Check sheet for the modelled part. Datum: model origin and axes. Units: mm. A direction names the side the tool comes from. Give positions to 0.01 mm unless a question says otherwise; leave off trailing zeros. Write each loop counter-clockwise with the first axis right and the second up, starting at its lowest first coordinate (ties: lowest second). Pieces come first, ordered by that corner, then holes. Notation, with made-up numbers: M 4,-33.5 L 39,-33.5 A27 cw 39,-16.5 Z; hole C 86,-31 d7. An arc over 180 degrees is marked long. Write item = value, one per line. Start each with the question number.
1) Mould release check, pull along Z, two halves, no side actions. Record for faces 1 (the cylindrical face through (48.89, -47.76, 69.79)), 2 (the cylindrical face through (-59.94, 2.64, 37.33)), 3 (the conical face through (-0.03, 60.74, 60.89)): released by +Z, released by -Z, zero draft, split by the parting line, or undercut.
2) Cross-section at C-C, the plane z = 76. Record the cut outline in (x, y).
3) Cross-section at B-B, the plane x = 75. Record the cut outline in (y, z), plus the area to 3 significant figures.
4) Cross-section at A-A, the plane z = 8. Record the cut outline in (x, y), plus the area to 3 significant figures.
5) Access from +Z, -Z, +X, -X, +Y, -Y to the whole of each face (thin tool, end or side, straight path). Record for faces 4 (the cylindrical face through (-48.89, 47.76, 69.79)), 5 (the cylindrical face through (-47.76, -48.89, 69.79)), 6 (the flat face through (46.5, 46.5, 55)), 7 (the cylindrical face through (55.946, 1.277, 74.154)).
6) Scan lines: line 1 along Y through (x, z) = (75, 3); line 2 along X through (y, z) = (1.5, 73) (1 decimal); line 3 along Y through (x, z) = (0, 48). Record each from-to range of solid material in increasing order. Write a range as [from, to].
7) Go/stop test with flat-tipped pins: pin 1 (2 mm diameter, centred on x = 8.5, z = 58, fed in from +Y); pin 2 (6 mm diameter, centred on y = 7, z = 58.5, fed in from -X); pin 3 (10 mm diameter, centred on y = -6, z = 64.5, fed in from +X). Record where each tip stops, or that it passes through.
```python
from build123d import *

# Parameters (mm, degrees)
SKETCH_1_R               = 5.25
EXTRUDE_1_DEPTH          = 15
SKETCH_2_R               = 60
EXTRUDE_2_DEPTH          = 40
EXTRUDE_3_DEPTH          = 30
PATTERN_CIRCULAR_1_COUNT = 4
FILLET_1_R               = 10
FILLET_2_R               = 5
SKETCH_6_R               = 35
CUT_EXTRUDE_1_DEPTH      = 154.05227865
SKETCH_7_R               = 45
CUT_EXTRUDE_2_DEPTH      = 20


with BuildPart() as part:
    # 草图1 → 凸台-拉伸1 (new body)
    with BuildSketch(Plane.XY):
        with BuildLine():
            Line((-80, 90), (80, 90))
            ThreePointArc((80, 90), (87.071067812, 87.071067812), (90, 80))
            Line((90, 80), (90, -80))
            ThreePointArc((90, -80), (87.071067812, -87.071067812), (80, -90))
            Line((80, -90), (-80, -90))
            ThreePointArc((-80, -90), (-87.071067812, -87.071067812), (-90, -80))
            Line((-90, -80), (-90, 80))
            ThreePointArc((-90, 80), (-87.071067812, 87.071067812), (-80, 90))
        make_face()
        with Locations((-75, 75)):
            Circle(SKETCH_1_R, mode=Mode.SUBTRACT)
        with Locations((75, 75)):
            Circle(SKETCH_1_R, mode=Mode.SUBTRACT)
        with Locations((-75, -75)):
            Circle(SKETCH_1_R, mode=Mode.SUBTRACT)
        with Locations((75, -75)):
            Circle(SKETCH_1_R, mode=Mode.SUBTRACT)
    extrude(amount=EXTRUDE_1_DEPTH)

    # 草图2 → 凸台-拉伸2 (add)
    with BuildSketch(Plane.XY.offset(15)):
        Circle(SKETCH_2_R)
    extrude(amount=EXTRUDE_2_DEPTH)

    # 草图3 → 凸台-拉伸3 (add)
    with BuildSketch(Plane.XY.offset(55)):
        with BuildLine():
            ThreePointArc((0, 77.781745931), (48.328171063, 48.328171063), (77.781745931, 0))
            ThreePointArc((77.781745931, 0), (48.328171063, -48.328171063), (0, -77.781745931))
            ThreePointArc((0, -77.781745931), (-48.328171063, -48.328171063), (-77.781745931, 0))
            ThreePointArc((-77.781745931, 0), (-48.328171063, 48.328171063), (0, 77.781745931))
        make_face()
    extrude(amount=EXTRUDE_3_DEPTH)

    # 草图5 → M10 螺纹孔1 (revolve, cut)
    with BuildSketch(Plane(origin=(0, 60, 85), x_dir=(0, -1, 0), z_dir=(1, 0, 0))):
        Polygon((0, 0), (0, 24.553657631), (4.25, 22), (4.25, 0), align=None)
    hole_wizard_m10_1 = revolve(axis=Axis((0, 60, 91.35), (0, 0, -1)), mode=Mode.SUBTRACT)

    # 阵列(圆周)1: M10 螺纹孔1 ×4 about axis
    pattern_circular_1_axis = Axis((0, 0, 0), (0, 0, 1))
    for i in range(1, PATTERN_CIRCULAR_1_COUNT):
        add(hole_wizard_m10_1.rotate(pattern_circular_1_axis, i * 360 / PATTERN_CIRCULAR_1_COUNT), mode=Mode.SUBTRACT)

    # 圆角1
    fillet_1_edges = [part.edges().sort_by_distance(p)[0] for p in [
        (-60, 0, 15),
    ]]
    fillet(fillet_1_edges, radius=FILLET_1_R)

    # 圆角2
    fillet_2_edges = [part.edges().sort_by_distance(p)[0] for p in [
        (-60, 0, 55),
    ]]
    fillet(fillet_2_edges, radius=FILLET_2_R)

    # 草图6 → 切除-拉伸1 (cut, through all)
    with BuildSketch(Plane.XY.offset(85)):
        Circle(SKETCH_6_R)
    extrude(amount=-CUT_EXTRUDE_1_DEPTH, mode=Mode.SUBTRACT)

    # 草图7 → 切除-拉伸2 (cut)
    with BuildSketch(Plane.XY.offset(85)):
        Circle(SKETCH_7_R)
    extrude(amount=-CUT_EXTRUDE_2_DEPTH, mode=Mode.SUBTRACT)


solid = part.part
```
Reply:
q1.face_1 = zero draft
q1.face_2 = undercut
q1.face_3 = released by +Z
q2.outline = M -77.78,0 A120 ccw 0,-77.78 A120 ccw 77.78,0 A120 ccw 0,77.78 A120 ccw Z; hole C -60,0 d8.5; hole C 0,0 d90; hole C 0,-60 d8.5; hole C 0,60 d8.5; hole C 60,0 d8.5
q3.outline = M -90,0 L -80.25,0 L -80.25,15 L -90,15 Z; M -69.75,0 L 69.75,0 L 69.75,15 L -69.75,15 Z; M -7.77,55 L 7.77,55 L 7.77,85 L -7.77,85 Z; M 80.25,0 L 90,0 L 90,15 L 80.25,15 Z
q3.area = 2,850 mm2
q4.outline = M -90,-80 A10 ccw -80,-90 L 80,-90 A10 ccw 90,-80 L 90,80 A10 ccw 80,90 L -80,90 A10 ccw -90,80 Z; hole C -75,-75 d10.5; hole C -75,75 d10.5; hole C 0,0 d70; hole C 75,-75 d10.5; hole C 75,75 d10.5
q4.area = 28,100 mm2
q5.face_4 = +Z, -X, +Y
q5.face_5 = +Z, -X, -Y
q5.face_6 = none
q5.face_7 = +Z
q6.line_1 = [-90, -80.25], [-69.75, 69.75], [80.25, 90]
q6.line_2 = [-77.3, -64], [-56, -45], [45, 56], [64, 77.3]
q6.line_3 = [-60, -35], [35, 60]
q7.pin_1 = 75.11
q7.pin_2 = -76.43
q7.pin_3 = 77.46
